Verification items for the finished model (mm, model axes). A direction names the side the tool comes from. Give positions to 0.01 mm unless a question says otherwise; leave off trailing zeros. Write each loop counter-clockwise with the first axis right and the second up, starting at its lowest first coordinate (ties: lowest second). Pieces come first, ordered by that corner, then holes. Notation, with made-up numbers: (52.5, 13) - (82.5, 13) arc R23 cw to (82.5, 46) - close; hole circle Ø6 at (85, -15). An arc over 180 degrees is marked (long way). Put each result on its own line as item: value.
from build123d import *

# Parameters (mm, degrees)
EXTRUDE_1_DEPTH = 2.5


with BuildPart() as part:
    # 草图1 → 凸台-拉伸1 (new, symmetric)
    with BuildSketch(Plane.XY):
        Polygon((0, 0), (0, 2.5), (-12, 2.5), (-12, 12.5), (-21, 12.5), (-21, -12.5), (-12, -12.5), (-12, -2.5), (0, -2.5), align=None)
        with BuildLine():
            Line((-18, -8), (-18, 8))
            ThreePointArc((-18, 8), (-16.5, 9.5), (-15, 8))
            Line((-15, 8), (-15, -8))
            ThreePointArc((-15, -8), (-16.5, -9.5), (-18, -8))
        make_face(mode=Mode.SUBTRACT)
    extrude(amount=EXTRUDE_1_DEPTH, both=True)


solid = part.part
Q1. Scan lines: line 1 along X through (y, z) = (4.25, 1.25); line 2 along X through (y, z) = (1.5, 2); line 3 along Y through (x, z) = (-2, 1). Record each from-to range of solid material in increasing order.
Answers follow:
line 1: x = -21 to -18, -15 to -12
line 2: x = -21 to -18, -15 to 0
line 3: y = -2.5 to 2.5
Q2. Section check B-B, the plane x = -16.5. Record the cut outline in (y, z), plus the area to 3 significant figures.
Answers follow:
outline: (-12.5, -2.5) - (-9.5, -2.5) - (-9.5, 2.5) - (-12.5, 2.5) - close; (9.5, -2.5) - (12.5, -2.5) - (12.5, 2.5) - (9.5, 2.5) - close
area: 30.0 mm2
Q3. Section check A-A, the plane y = 3.25. Record the cut outline in (x, z).
Answers follow:
outline: (-21, -2.5) - (-18, -2.5) - (-18, 2.5) - (-21, 2.5) - close; (-15, -2.5) - (-12, -2.5) - (-12, 2.5) - (-15, 2.5) - close
Q4. Section check D-D, the plane x = -8.5. Record the cut outline in (y, z).
Answers follow:
outline: (-2.5, -2.5) - (2.5, -2.5) - (2.5, 2.5) - (-2.5, 2.5) - close
Q5. Set-up check for faces 4 (the face through (-12, -8, 0)), 5 (the face through (-18, 0, 0)), 6 (the face through (-14, 1, 2.5)), 7 (the face through (-21, 0, 0)), 8 (the face through (-12, 7, 0)): record each of +Z, -Z, +X, -X, +Y, -Y from which the full face is reachable in a straight line by a thin tool's end or side.
Answers follow:
face 4: +Z, -Z, +X, -Y
face 5: +Z, -Z
face 6: +Z, +X, -X, +Y, -Y
face 7: +Z, -Z, -X, +Y, -Y
face 8: +Z, -Z, +X, +Y
Q6. Go/stop test with flat-tipped pins: pin 1 Ø1 at (x, y) = (-9, 3.5) entering from -Z; pin 2 Ø1.5 at (x, z) = (-3, 1) entering from +Y; pin 3 Ø1.5 at (x, z) = (-8, 0.5) entering from -Y. Record where each tip stops, or that it passes through.
Answers follow:
pin 1: passes through
pin 2: stops at y = 2.5
pin 3: stops at y = -2.5
Q7. Release check for a two-part mould opening along X. For faces 1 (the face through (-16.5, 9.5, 0)), 2 (the face through (-6, 2.5, 0)), 3 (the face through (0, 0, 0)) record: released by +X, released by -X, zero draft, split by the parting line, or undercut.
Answers follow:
face 1: undercut
face 2: zero draft
face 3: released by +X
Q8. Section check C-C, the plane z = -2.1. Record the cut outline in (x, y).
Answers follow:
outline: (-21, -12.5) - (-12, -12.5) - (-12, -2.5) - (0, -2.5) - (0, 2.5) - (-12, 2.5) - (-12, 12.5) - (-21, 12.5) - close; hole (-18, -8) arc R1.5 ccw to (-15, -8) - (-15, 8) arc R1.5 ccw to (-18, 8) - close
